Design review of the part built by this model. Coordinates are the model's own, in mm. Face numbers are marked on the shaded views. A direction names the side the tool comes from. Round coordinates to 2 decimals unless told otherwise and drop trailing zeros. Loops run counter-clockwise (first coordinate to the right, second up) from the corner with the lowest first, then second, coordinate; pieces in that order, holes last. Notation, with made-up numbers: (37.25, 30) - (82.25, 30) arc R4 cw to (82.25, 37) - close; hole circle Ø6 at (61.25, 10.5). An arc over 180 degrees is marked (long way). Use one line per item in the form item = value. Start each with the question number.
(1) We need section D-D, the plane y = -6. Write out the cut boundary in (x, z).
(2) The part is to be moulded in two halves that separate along Y. For the marked faces 4, 5 and 6, say which applies: released by +Y, released by -Y, zero draft, split by the parting line, or undercut.
(3) Wall thickness on probe 1 along X at (y, z) = (-13, 10); probe 2 along Z at (x, y) = (-15, 19.75); probe 3 along Y at (x, z) = (-11, 3.5): over which ranges is each line inside the solid? List them lowest first. Write a range as [from, to].
(4) We need section C-C, the plane x = -8.5. Write out the cut boundary in (y, z), then the cut area to 3 significant figures.
(5) We need section B-B, the plane x = 5. Write out the cut boundary in (y, z).
(6) For pin 1 (1.2 mm diameter, centred on x = 18, z = 8, fed in from +Y); pin 2 (4.5 mm diameter, centred on x = 17.5, z = 7, fed in from -Y); pin 3 (8 mm diameter, centred on x = -15, z = 10, fed in from -Y), all flat-tipped, find the tip position at first contact; note any pin that passes through.
(7) We need section A-A, the plane z = 10. Write out the cut boundary in (x, y), then the cut area to 3 significant figures.
(8) Machinability: for the marked faces 1, 2 and 3, which of the approach directions +Z, -Z, +X, -X, +Y, -Y give a long, thin tool a straight path to every point of the face, cutting with its end or side? Answer none if there is none.
from build123d import *

# Parameters (mm, degrees)
SKETCH_1_W          = 50
SKETCH_1_H          = 50
SKETCH_1_R          = 10
EXTRUDE_1_DEPTH     = 20
CHAMFER_1_SIZE      = 10
CHAMFER_2_SIZE      = 1
HOLE_WIZARD_M8_1_D  = 6.8
SKETCH_5_R          = 4.5
CUT_EXTRUDE_1_DEPTH = 30
SKETCH_6_W          = 34.59440866
SKETCH_6_H          = 2
CUT_EXTRUDE_2_DEPTH = 44
SKETCH_7_R          = 5
CUT_EXTRUDE_5_DEPTH = 26


with BuildPart() as part:
    # 草图1 → 凸台-拉伸1 (new body)
    with BuildSketch(Plane.XY):
        Rectangle(SKETCH_1_W, SKETCH_1_H)
        with Locations((5, 5)):
            Circle(SKETCH_1_R, mode=Mode.SUBTRACT)
    extrude(amount=EXTRUDE_1_DEPTH)

    # 倒角1
    chamfer_1_edges = [part.edges().sort_by_distance(p)[0] for p in [
        (25, -25, 10),
        (-25, 25, 10),
        (25, 25, 10),
    ]]
    chamfer(chamfer_1_edges, length=CHAMFER_1_SIZE)

    # 倒角2
    chamfer_2_edges = [part.edges().sort_by_distance(p)[0] for p in [
        (-25, -25, 10),
    ]]
    chamfer(chamfer_2_edges, length=CHAMFER_2_SIZE)

    # M8 螺纹孔1 (through all)
    with Locations(Plane(origin=(0, 25, 0), x_dir=(1, 0, 0), z_dir=(0, 1, 0))):
        with Locations((-15, -10)):
            Hole(HOLE_WIZARD_M8_1_D / 2)

    # 草图5 → 切除-拉伸1 (cut)
    with BuildSketch(Plane.XZ.offset(25)):
        with Locations(Location((-15, 10, 0), (0, 0, 270))):
            Circle(SKETCH_5_R)
    extrude(amount=-CUT_EXTRUDE_1_DEPTH, mode=Mode.SUBTRACT)

    # 草图6 → 切除-拉伸2 (cut)
    with BuildSketch(Plane.ZY.offset(25)):
        with Locations((10, 5)):
            Rectangle(SKETCH_6_W, SKETCH_6_H)
    extrude(amount=-CUT_EXTRUDE_2_DEPTH, mode=Mode.SUBTRACT)

    # 草图7 → 切除-拉伸5 (cut)
    with BuildSketch(Plane.XZ.offset(25)):
        with Locations(Location((5, 10, 0), (0, 0, 270))):
            Circle(SKETCH_7_R)
    extrude(amount=-CUT_EXTRUDE_5_DEPTH, mode=Mode.SUBTRACT)


solid = part.part
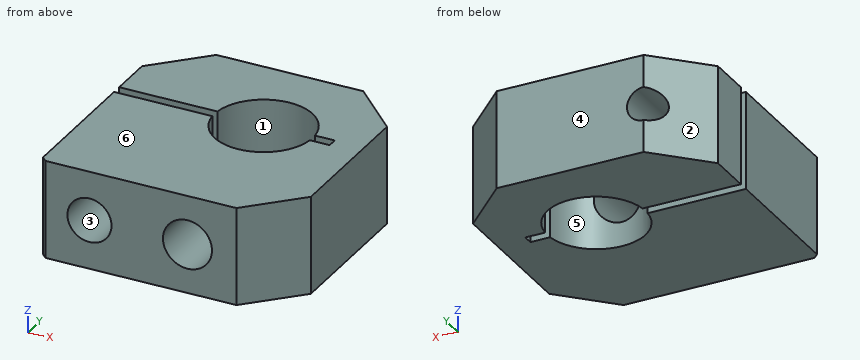
Data:
q1.outline = (-25, 0) - (25, 0) - (25, 20) - (-25, 20) - close; hole circle Ø9 at (-15, 10); hole circle Ø10 at (5, 10)
q2.face_4 = released by +Y
q2.face_5 = undercut
q2.face_6 = zero draft
q3.probe_1 = [-25, -19.5], [-10.5, 0], [10, 25]
q3.probe_2 = [0, 6.6], [13.4, 20]
q3.probe_3 = [-25, 4], [6, 25]
q4.outline = (-25, 0) - (4, 0) - (4, 20) - (-25, 20) - close; (6, 0) - (25, 0) - (25, 20) - (6, 20) - close
q4.area = 960 mm^2
q5.outline = (-25, 0) - (-5, 0) - (-5, 5) - (-25, 5) - close; (-25, 15) - (-5, 15) - (-5, 20) - (-25, 20) - close; (15, 0) - (25, 0) - (25, 20) - (15, 20) - close
q6.pin_1 = 22.6
q6.pin_2 = -24.75
q6.pin_3 = 6
q7.outline = (-25, -24) - (-24, -25) - (-19.5, -25) - (-19.5, 4) - (-25, 4) - close; (-25, 6) - (-18.4, 6) - (-18.4, 21.6) - (-25, 15) - close; (-11.6, 6) - (-4.95, 6) arc R10 cw to (14.95, 6) - (19, 6) - (19, 4) - (14.95, 4) arc R10 cw to (10, -3.66) - (10, -25) - (15, -25) - (25, -15) - (25, 15) - (15, 25) - (-11.6, 25) - close; (-10.5, -25) - (0, -25) - (0, -3.66) arc R10 cw to (-4.95, 4) - (-10.5, 4) - close
q7.area = 1,400 mm^2
q8.face_1 = +Z, -Z
q8.face_2 = +Z, -Z, -X, +Y
q8.face_3 = -Y
